Build history of the part. All positions in model axes, mm. Round coordinates to 2 decimals unless told otherwise and drop trailing zeros. Write each loop counter-clockwise with the first axis right and the second up, starting at its lowest first coordinate (ties: lowest second). Pieces come first, ordered by that corner, then holes.
Item 1: Band-saw the part on B-B, the plane x = -442. Write the cut outline in (y, z), then the cut area to 3 significant figures.
Item 2: Wall check: probe 1 along X at (y, z) = (-1.95, 1.5); probe 2 along Y at (x, z) = (637, 2.5); probe 3 along Y at (x, z) = (-383, 0.5). Give the ranges that are in metal, low to high.
Item 3: Drop flat-ended pins along their axis: pin 1 Ø1.1 at (x, z) = (440.5, 0.5) entering from -Y; pin 2 Ø1 at (x, y) = (228, 0) entering from +Z. Give the stop position or say it passes through.
Item 4: Band-saw the part on A-A, the plane z = 4.5. Write the cut outline in (x, y).
Item 5: Band-saw the part on C-C, the plane y = -0.6. Write the cut outline in (x, z).
Item 6: Band-saw the part on D-D, the plane x = -92. Write the cut outline in (y, z), then the cut area to 3 significant figures.
```python
from build123d import *

# Parameters (mm, degrees)
SKETCH_1_W               = 1390
SKETCH_1_H               = 5
SKETCH_1_W_2             = 1388
SKETCH_1_H_2             = 3
EXTRUDE_1_DEPTH          = 10
SKETCH_2_W               = 1
SKETCH_2_H               = 5
EXTRUDE_1_2_DEPTH        = 1389
CUT_EXTRUDE_1_DEPTH      = 1390.038246414
CUT_EXTRUDE_1_DEPTH_BACK = 1390.038246414
SKETCH_3_W               = 9
SKETCH_3_H               = 3
CUT_EXTRUDE_START        = -325
SKETCH_4_W               = 10
SKETCH_4_H               = 1
CUT_EXTRUDE_2_DEPTH      = 102
SKETCH_5_W               = 6
SKETCH_5_H               = 9
CUT_EXTRUDE_5_DEPTH      = 4


with BuildPart() as part:
    # 草图1 → Extrude 1 (new body)
    with BuildSketch(Plane.XY):
        Rectangle(SKETCH_1_W, SKETCH_1_H)
        Rectangle(SKETCH_1_W_2, SKETCH_1_H_2, mode=Mode.SUBTRACT)
    extrude(amount=EXTRUDE_1_DEPTH)

    # 草图2 → Extrude 1 2 (add)
    with BuildSketch(Plane.ZY.offset(695)):
        with Locations((0.5, 0)):
            Rectangle(SKETCH_2_W, SKETCH_2_H)
    extrude(amount=-EXTRUDE_1_2_DEPTH)

    # 草图3 → 切除-拉伸1 (cut, two sides: drawn at the far end of the back side and taken through both)
    with BuildSketch(Plane.ZY.offset(-694).offset(-CUT_EXTRUDE_1_DEPTH_BACK)):
        with Locations((5.5, 0)):
            Rectangle(SKETCH_3_W, SKETCH_3_H)
    extrude(amount=CUT_EXTRUDE_1_DEPTH + CUT_EXTRUDE_1_DEPTH_BACK, mode=Mode.SUBTRACT)

    # 草图4 → 切除-拉伸2 (cut)
    with BuildSketch(Plane.ZY.offset(695).offset(CUT_EXTRUDE_START)):
        with Locations((5, -2)):
            Rectangle(SKETCH_4_W, SKETCH_4_H)
    cut_extrude_2 = extrude(amount=CUT_EXTRUDE_2_DEPTH, mode=Mode.SUBTRACT)

    # 镜向1: 切除-拉伸2 across plane
    add(cut_extrude_2.mirror(Plane(origin=(0, 0, 0), x_dir=(0, 0, 1), z_dir=(1, 0, 0))), mode=Mode.SUBTRACT)

    # 草图5 → 切除-拉伸5 (cut)
    with BuildSketch(Plane.XZ.offset(2.5)):
        with Locations((475, 5.5)):
            Rectangle(SKETCH_5_W, SKETCH_5_H)
    extrude(amount=-CUT_EXTRUDE_5_DEPTH, mode=Mode.SUBTRACT)


solid = part.part
```
Results:
1. outline: (-1.5, 0) - (2.5, 0) - (2.5, 10) - (1.5, 10) - (1.5, 1) - (-1.5, 1) - close
1. area: 13.0 mm2
2. probe 1: x = -695 to -472, -370 to 370, 478 to 695
2. probe 2: y = -2.5 to -1.5, 1.5 to 2.5
2. probe 3: y = -1.5 to 2.5
3. pin 1: stops at y = -1.5
3. pin 2: stops at z = 1
4. outline: (-695, -2.5) - (-472, -2.5) - (-472, -1.5) - (-695, -1.5) - close; (-695, 1.5) - (695, 1.5) - (695, 2.5) - (-695, 2.5) - close; (-370, -2.5) - (370, -2.5) - (370, -1.5) - (-370, -1.5) - close; (478, -2.5) - (695, -2.5) - (695, -1.5) - (478, -1.5) - close
5. outline: (-695, 0) - (695, 0) - (695, 1) - (-695, 1) - close
6. outline: (-2.5, 0) - (2.5, 0) - (2.5, 10) - (1.5, 10) - (1.5, 1) - (-1.5, 1) - (-1.5, 10) - (-2.5, 10) - close
6. area: 23.0 mm2
